The drawing under review shows one solid part. Ordinate dimensions are in mm from its lowest x, y, z. Give positions to 0.01 mm unless a question says otherwise; leave off trailing zeros. Write each loop counter-clockwise with the first axis right and the second up, starting at its lowest first coordinate (ties: lowest second). Pieces come first, ordered by that corner, then holes. Notation, with made-up numbers: M 20,75.5 L 70,75.5 A17 ccw 70,80.5 Z; hole C -32.5,85.5 d6. An arc over 180 degrees is marked long. Write each question's results on one line, items separated by ' | '. Start each with the question number.
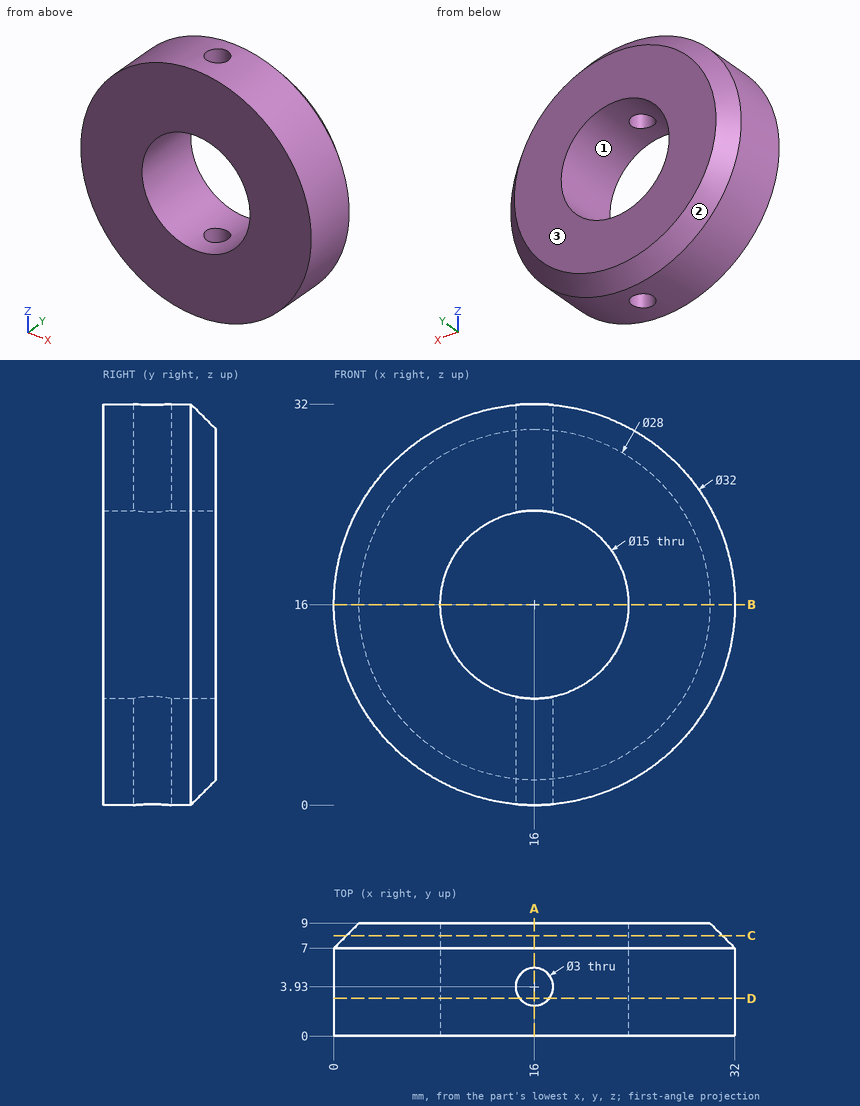
Q1. Wall thickness on line 1 along X through (y, z) = (8, 18) (1 decimal); line 2 along X through (y, z) = (8.5, 11); line 3 along Z through (x, y) = (12, 3.5) (1 decimal): over which ranges is each line inside the solid? List them lowest first. Write a range as from..to.
Q2. We need section D-D on y = 3. Write out the cut boundary in (x, z).
Q3. We need section B-B on z = 16. Write out the cut boundary in (x, y), and give its area (3 significant figures).
Q4. We need section A-A on x = 16. Write out the cut boundary in (y, z).
Q5. For pin 1 Ø2 at (x, y) = (26, 6) entering from -Z, flat-tipped, find the tip position at first contact; note if it passes through.
Q6. The part is to be moulded in two halves that separate along Z. For the marked faces 1, 2 and 3, say which applies: pulls with the +Z half, pulls with the -Z half, needs draft (parallel to the pull), parting line crosses it, or undercut.
Q7. We need section C-C on y = 8. Write out the cut boundary in (x, z).
Answer sheet:
1) line 1: 1.1..8.8, 23.2..30.9 | line 2: 2.39..10.41, 21.59..29.61 | line 3: 0.5..9.7, 22.3..31.5
2) outline: M 14.82,0.04 L 14.82,8.59 A7.5 cw 14.82,23.41 L 14.82,31.96 A16 ccw Z; M 17.18,0.04 A16 ccw 17.18,31.96 L 17.18,23.41 A7.5 cw 17.18,8.59 Z
3) outline: M 0,0 L 8.5,0 L 8.5,9 L 2,9 L 0,7 Z; M 23.5,0 L 32,0 L 32,7 L 30,9 L 23.5,9 Z | area: 149 mm^2
4) outline: M 0,0 L 2.43,0 L 2.43,8.5 L 0,8.5 Z; M 0,23.5 L 2.43,23.5 L 2.43,32 L 0,32 Z; M 5.43,0 L 7,0 L 9,2 L 9,8.5 L 5.43,8.5 Z; M 5.43,23.5 L 9,23.5 L 9,30 L 7,32 L 5.43,32 Z
5) pin 1: z = 2.77
6) face 1: undercut | face 2: parting line crosses it | face 3: needs draft
7) outline: C 16,16 d30; hole C 16,16 d15
